from build123d import *

# Parameters (mm, degrees)
SKETCH_1_W               = 102
SKETCH_1_H               = 12
CUT_EXTRUDE_1_DEPTH      = 83
M6X1_0_1_AT_2_COUNT      = 2
M6X1_0_1_AT_2_PITCH      = 50
PATTERN_CIRCULAR_1_COUNT = 8
SKETCH_7_R               = 1.65
CUT_EXTRUDE_2_DEPTH      = 30
SKETCH_8_R               = 4
CUT_EXTRUDE_3_DEPTH      = 7
PATTERN_CIRCULAR_2_COUNT = 4


with BuildPart() as part:
    # 草图1 → 旋转1 (revolve)
    with BuildSketch(Plane.XY, mode=Mode.PRIVATE) as revolve_1_sk:
        with Locations((69, 0)):
            Rectangle(SKETCH_1_W, SKETCH_1_H)
    revolve(revolve_1_sk.sketch.rotate(Axis((0, 0, 0), (0, 1, 0)), 90), axis=Axis((0, 0, 0), (0, 1, 0)))

    # 草图4 → 切除-拉伸1 (cut)
    with BuildSketch(Plane(origin=(0, 6, 0), x_dir=(1, 0, 0), z_dir=(0, 1, 0))):
        Polygon((110, 627.554648283), (110, 47.958315233), (110, -47.958315233), (110, -627.554648283), (1269.1926661, -627.554648283), (1269.1926661, 627.554648283), align=None)
    cut_extrude_1 = extrude(amount=-CUT_EXTRUDE_1_DEPTH, mode=Mode.SUBTRACT)

    # 草图6 → M6x1.0 螺纹孔1 (revolve, cut)
    with BuildSketch(Plane(origin=(110, 0, 25), x_dir=(0, 0, -1), z_dir=(0, 1, 0))):
        Polygon((0, 0), (0, 13.502151548), (2.5, 12), (2.5, 0), align=None)
    m6x1_0_1 = revolve(axis=Axis((116.35, 0, 25), (-1, 0, 0)), mode=Mode.SUBTRACT)

    # M6x1.0 螺纹孔1 at 2: M6x1.0 螺纹孔1 ×2
    with Locations(*[(0, 0, -i * M6X1_0_1_AT_2_PITCH) for i in range(1, M6X1_0_1_AT_2_COUNT)]):
        add(m6x1_0_1, mode=Mode.SUBTRACT)

    # 阵列(圆周)1: 切除-拉伸1, M6x1.0 螺纹孔1 ×8 about axis
    pattern_circular_1_axis = Axis((0, 0, 0), (0, 1, 0))
    add([cut_extrude_1.rotate(pattern_circular_1_axis, i * 360 / PATTERN_CIRCULAR_1_COUNT) for i in range(1, PATTERN_CIRCULAR_1_COUNT)], mode=Mode.SUBTRACT)
    add([m6x1_0_1.rotate(pattern_circular_1_axis, i * 360 / PATTERN_CIRCULAR_1_COUNT) for i in range(1, PATTERN_CIRCULAR_1_COUNT)], mode=Mode.SUBTRACT)

    # 阵列(圆周)1 copy 1 sketch → 阵列(圆周)1 copy 1 (revolve, cut)
    with BuildSketch(Plane(origin=(60.104076401, 0, -95.45941546), x_dir=(-0.7071067811865475, 0, -0.7071067811865476), z_dir=(0, 1, 0))):
        Polygon((0, 0), (0, 13.502151548), (2.5, 12), (2.5, 0), align=None)
    revolve(axis=Axis((64.594204461, 0, -99.949543521), (-0.7071067811865476, 0, 0.7071067811865475)), mode=Mode.SUBTRACT)

    # 阵列(圆周)1 copy 2 sketch → 阵列(圆周)1 copy 2 (revolve, cut)
    with BuildSketch(Plane(origin=(-25, 0, -110), x_dir=(-1, 0, 0), z_dir=(0, 1, 0))):
        Polygon((0, 0), (0, 13.502151548), (2.5, 12), (2.5, 0), align=None)
    revolve(axis=Axis((-25, 0, -116.35), (0, 0, 1)), mode=Mode.SUBTRACT)

    # 阵列(圆周)1 copy 3 sketch → 阵列(圆周)1 copy 3 (revolve, cut)
    with BuildSketch(Plane(origin=(-95.45941546, 0, -60.104076401), x_dir=(-0.7071067811865476, 0, 0.7071067811865475), z_dir=(0, 1, 0))):
        Polygon((0, 0), (0, 13.502151548), (2.5, 12), (2.5, 0), align=None)
    revolve(axis=Axis((-99.949543521, 0, -64.594204461), (0.7071067811865475, 0, 0.7071067811865476)), mode=Mode.SUBTRACT)

    # 阵列(圆周)1 copy 4 sketch → 阵列(圆周)1 copy 4 (revolve, cut)
    with BuildSketch(Plane(origin=(-110, 0, 25), x_dir=(0, 0, 1), z_dir=(0, 1, 0))):
        Polygon((0, 0), (0, 13.502151548), (2.5, 12), (2.5, 0), align=None)
    revolve(axis=Axis((-116.35, 0, 25), (1, 0, 0)), mode=Mode.SUBTRACT)

    # 阵列(圆周)1 copy 5 sketch → 阵列(圆周)1 copy 5 (revolve, cut)
    with BuildSketch(Plane(origin=(-60.104076401, 0, 95.45941546), x_dir=(0.7071067811865475, 0, 0.7071067811865477), z_dir=(0, 1, 0))):
        Polygon((0, 0), (0, 13.502151548), (2.5, 12), (2.5, 0), align=None)
    revolve(axis=Axis((-64.594204461, 0, 99.949543521), (0.7071067811865477, 0, -0.7071067811865475)), mode=Mode.SUBTRACT)

    # 阵列(圆周)1 copy 6 sketch → 阵列(圆周)1 copy 6 (revolve, cut)
    with BuildSketch(Plane(origin=(25, 0, 110), x_dir=(1, 0, 0), z_dir=(0, 1, 0))):
        Polygon((0, 0), (0, 13.502151548), (2.5, 12), (2.5, 0), align=None)
    revolve(axis=Axis((25, 0, 116.35), (0, 0, -1)), mode=Mode.SUBTRACT)

    # 阵列(圆周)1 copy 7 sketch → 阵列(圆周)1 copy 7 (revolve, cut)
    with BuildSketch(Plane(origin=(95.45941546, 0, 60.104076401), x_dir=(0.7071067811865477, 0, -0.7071067811865474), z_dir=(0, 1, 0))):
        Polygon((0, 0), (0, 13.502151548), (2.5, 12), (2.5, 0), align=None)
    revolve(axis=Axis((99.949543521, 0, 64.594204461), (-0.7071067811865474, 0, -0.7071067811865477)), mode=Mode.SUBTRACT)

    # 草图7 → 切除-拉伸2 (cut)
    with BuildSketch(Plane(origin=(0, 6, 0), x_dir=(1, 0, 0), z_dir=(0, 1, 0))):
        with Locations(Location((18.384776311, 18.384776311, 0), (0, 0, 270))):
            Circle(SKETCH_7_R)
    cut_extrude_2 = extrude(amount=-CUT_EXTRUDE_2_DEPTH, mode=Mode.SUBTRACT)

    # 草图8 → 切除-拉伸3 (cut)
    with BuildSketch(Plane(origin=(0, 6, 0), x_dir=(1, 0, 0), z_dir=(0, 1, 0))):
        with Locations(Location((18.384776311, 18.384776311, 0), (0, 0, 270))):
            Circle(SKETCH_8_R)
    cut_extrude_3 = extrude(amount=-CUT_EXTRUDE_3_DEPTH, mode=Mode.SUBTRACT)

    # 阵列(圆周)2: 切除-拉伸2, 切除-拉伸3 ×4 about axis
    pattern_circular_2_axis = Axis((0, 0, 0), (0, 1, 0))
    add([cut_extrude_2.rotate(pattern_circular_2_axis, i * 360 / PATTERN_CIRCULAR_2_COUNT) for i in range(1, PATTERN_CIRCULAR_2_COUNT)], mode=Mode.SUBTRACT)
    add([cut_extrude_3.rotate(pattern_circular_2_axis, i * 360 / PATTERN_CIRCULAR_2_COUNT) for i in range(1, PATTERN_CIRCULAR_2_COUNT)], mode=Mode.SUBTRACT)


solid = part.part
CAD build for the part. Positions are in the model's coordinates, mm. A direction names the side the tool comes from. Round coordinates to 2 decimals unless told otherwise and drop trailing zeros. Loops run counter-clockwise (first coordinate to the right, second up) from the corner with the lowest first, then second, coordinate; pieces in that order, holes last.
(1) Cut at D-D (x = 70). Give the cut face in (y, z).
(2) Wall check: line 1 along Y through (x, z) = (25, 100.5); line 2 along Z through (x, y) = (-54, -1); line 3 along Z through (x, y) = (-107, 0). Give the ranges that are in metal, low to high.
(3) Cut at B-B (z = 1). Give the cut face in (x, y).
(4) Drop flat-ended pins along their axis: pin 1 (4.5 mm diameter, centred on y = 0, z = 25, fed in from -X); pin 2 (7 mm diameter, centred on x = 18.38, z = 18.38, fed in from +Y); pin 3 (3 mm diameter, centred on y = -1.5, z = 79, fed in from -X). Give the stop position or say it passes through.
(5) Which spindle directions (+Z, -Z, +X, -X, +Y, -Y) get a long thin tool onto all of the face, cutting with end or side? Do faces 5 (the cylindrical face through (-26.84, -1.69, 104.08)), 6 (the cylindrical face through (18.91, 2.55, 22.35)), 7 (the conical face through (96.76, 0.17, -25.4)). Say none if no direction does.
(6) Cut at A-A (x = 0). Give the cut face in (y, z).
(7) Cut at C-C (z = 66). Give the cut face in (x, y), plus the area to 3 significant figures.
(8) Two-plate mould, pull along Z, no slides. Class faces 1 (the flat face through (77.331, 0.084, -78.233)), 2 (the conical face through (25.4, 0.17, 96.76)), 3 (the conical face through (-96.76, 0.17, 25.4)), 4 (the cylindrical face through (-22.5, -0.1, -104.1)): +Z half, -Z half, draft (parallel to the pull), parting line (faces both ways), or undercut.
Findings below:
1. outline: (-6, -85.56) - (6, -85.56) - (6, 85.56) - (-6, 85.56) - close
2. line 1: y = -6 to -2.5, 2.5 to 6
2. line 2: z = -101.56 to -92.6, -86.11 to 86.11, 92.6 to 101.56
2. line 3: z = -48.56 to -27.5, -22.5 to 22.5, 27.5 to 48.56
3. outline: (-110, -6) - (-17.97, -6) - (-17.97, 6) - (-110, 6) - close; (17.97, -6) - (110, -6) - (110, 6) - (17.97, 6) - close
4. pin 1: stops at x = -97.85
4. pin 2: stops at y = -1
4. pin 3: stops at x = -78.06
5. face 5: +Z
5. face 6: +Y
5. face 7: +X
6. outline: (-6, -110) - (6, -110) - (6, -18) - (-6, -18) - close; (-6, 18) - (6, 18) - (6, 110) - (-6, 110) - close
7. outline: (-89.56, -6) - (89.56, -6) - (89.56, 6) - (-89.56, 6) - close
7. area: 2,150 mm2
8. face 1: -Z half
8. face 2: +Z half
8. face 3: undercut
8. face 4: draft
